Build history of the part. All positions in model axes, mm. A direction names the side the tool comes from. Round coordinates to 2 decimals unless told otherwise and drop trailing zeros. Write each loop counter-clockwise with the first axis right and the second up, starting at its lowest first coordinate (ties: lowest second). Pieces come first, ordered by that corner, then holes. Notation, with made-up numbers: (20, 24.25) - (79, 24.25) arc R28 cw to (79, 55.25) - close; hole circle Ø1 at (44.5, 45.5). An arc over 180 degrees is marked (long way). Answer as a JSON object with one key per item and string values. Group by question number.
Item 1: Flat gauge pins, fed straight in: pin 1 (2 mm diameter, centred on x = 25, y = -3.5, fed in from +Z); pin 2 (6 mm diameter, centred on x = 2, y = -5.5, fed in from +Z); pin 3 (4 mm diameter, centred on x = -4, z = 22.5, fed in from +Y); pin 4 (1.5 mm diameter, centred on y = -5, z = 26, fed in from -X). Where does each tip first touch, or does it go through?
Item 2: Slice it at D-D, the plane x = -9.5. List the corners of the cut face in (y, z), then the cut area to 3 significant figures.
Item 3: Slice it at C-C, the plane x = -39. List the corners of the cut face in (y, z).
Item 4: Slice it at A-A, the plane z = 2. List the corners of the cut face in (x, y), then the cut area to 3 significant figures.
Item 5: Two-plate mould, pull along X, no slides. Class faces 5 (the flat face through (43, 0, 0)), 6 (the flat face through (41.15, 0, 0)), 7 (the cylindrical face through (-0.867, -3.905, 17.853)): +X half, -X half, draft (parallel to the pull), parting line (faces both ways), or undercut.
Item 6: Slice it at B-B, the plane y = 0. List the corners of the cut face in (x, z).
Item 7: Which spindle directions (+Z, -Z, +X, -X, +Y, -Y) get a long thin tool onto all of the face, cutting with end or side? Do faces 1 (the cylindrical face through (39.05, 7.15, -0.08)), 2 (the cylindrical face through (-0.867, -3.905, 29.993)), 3 (the cylindrical face through (3.796, -0.167, 28.993)), 4 (the flat face through (-1, -12, 0)). Say none if no direction does.
Item 8: Probe line 1 (Z direction, x = 18.5, y = -8); line 2 (X direction, y = 5, z = 6.5); line 3 (X direction, y = 2.5, z = 8). List the from-to ranges inside material, lowest first. Write a range as from..to.
from build123d import *

# Parameters (mm, degrees)
SKETCH_1_W          = 86
SKETCH_1_H          = 24
EXTRUDE_1_DEPTH     = 5.5
SKETCH_2_R          = 4
EXTRUDE_2_DEPTH     = 3.5
SKETCH_3_R          = 4
EXTRUDE_3_DEPTH     = 21.5
CUT_EXTRUDE_4_DEPTH = 58.349803836
SKETCH_15_R         = 4
CUT_EXTRUDE_5_DEPTH = 9.999
SKETCH_4_W          = 0.2
SKETCH_4_H          = 1
SKETCH_16_R         = 2.9995
EXTRUDE_4_DEPTH     = 8.999
SKETCH_18_R         = 6
EXTRUDE_5_DEPTH     = 2
SKETCH_22_R         = 7.5
EXTRUDE_7_DEPTH     = 11
CHAMFER_1_SIZE      = 1


with BuildPart() as part:
    # 草图1 → 凸台-拉伸1 (new, symmetric)
    with BuildSketch(Plane.XY):
        Rectangle(SKETCH_1_W, SKETCH_1_H)
    extrude(amount=EXTRUDE_1_DEPTH, both=True)

    # 草图2 → 凸台-拉伸2 (add)
    with BuildSketch(Plane.XY.offset(5.5)):
        Circle(SKETCH_2_R)
    extrude(amount=EXTRUDE_2_DEPTH)

    # 草图3 → 凸台-拉伸3 (add)
    with BuildSketch(Plane.XY.offset(9)):
        Circle(SKETCH_3_R)
    extrude(amount=EXTRUDE_3_DEPTH)

    # 草图14 → 切除-拉伸4 (cut, through all)
    with BuildSketch(Plane(origin=(0, 0, -5.5), x_dir=(-1, 0, 0), z_dir=(0, 0, -1))):
        with BuildLine():
            Line((-36.85, 5), (-36.85, -5))
            ThreePointArc((-36.85, -5), (-39, -7.15), (-41.15, -5))
            Line((-41.15, -5), (-41.15, 5))
            ThreePointArc((-41.15, 5), (-39, 7.15), (-36.85, 5))
        make_face()
        with BuildLine():
            Line((36.85, 5), (36.85, -5))
            ThreePointArc((36.85, -5), (39, -7.15), (41.15, -5))
            Line((41.15, -5), (41.15, 5))
            ThreePointArc((41.15, 5), (39, 7.15), (36.85, 5))
        make_face()
    extrude(amount=-CUT_EXTRUDE_4_DEPTH, mode=Mode.SUBTRACT)

    # 草图15 → 切除-拉伸5 (cut)
    with BuildSketch(Plane(origin=(0, 0, -5.5), x_dir=(-1, 0, 0), z_dir=(0, 0, -1))):
        with Locations(Location((0, 0, 0), (0, 0, 180))):
            Circle(SKETCH_15_R)
    extrude(amount=-CUT_EXTRUDE_5_DEPTH, mode=Mode.SUBTRACT)

    # 草图4 → 切除-旋转1 (revolve, cut)
    with BuildSketch(Plane(origin=(0, 0, 0), x_dir=(1, 0, 0), z_dir=(0, 1, 0))):
        with Locations((-3.9, -29)):
            Rectangle(SKETCH_4_W, SKETCH_4_H)
    revolve(axis=Axis((0, 0, 0), (0, 0, 1)), mode=Mode.SUBTRACT)

    # 草图16 → 凸台-拉伸4 (add)
    with BuildSketch(Plane(origin=(0, 0, 4.499), x_dir=(-1, 0, 0), z_dir=(0, 0, -1))):
        Circle(SKETCH_16_R)
    extrude(amount=EXTRUDE_4_DEPTH)

    # 草图18 → 凸台-拉伸5 (add)
    with BuildSketch(Plane.XY.offset(5.5)):
        Circle(SKETCH_18_R)
    extrude(amount=EXTRUDE_5_DEPTH)

    # 草图22 → 凸台-拉伸7 (add)
    with BuildSketch(Plane(origin=(0, 0, -5.5), x_dir=(-1, 0, 0), z_dir=(0, 0, -1))):
        Circle(SKETCH_22_R)
    extrude(amount=-EXTRUDE_7_DEPTH)

    # 倒角1
    chamfer_1_edges = [part.edges().sort_by_distance(p)[0] for p in [
        (43, -12, 0),
        (-43, -12, 0),
        (-43, 12, 0),
        (43, 12, 0),
    ]]
    chamfer(chamfer_1_edges, length=CHAMFER_1_SIZE)


solid = part.part
Geometry says:
{
 "1": {"pin 1": "stops at z = 5.5", "pin 2": "stops at z = 30.5", "pin 3": "stops at y = 3.46", "pin 4": "passes through"},
 "2": {"outline": "(-12, -5.5) - (12, -5.5) - (12, 5.5) - (-12, 5.5) - close", "area": "264 mm^2"},
 "3": {"outline": "(-12, -5.5) - (-7.15, -5.5) - (-7.15, 5.5) - (-12, 5.5) - close; (7.15, -5.5) - (12, -5.5) - (12, 5.5) - (7.15, 5.5) - close"},
 "4": {"outline": "(-43, -11) - (-42, -12) - (42, -12) - (43, -11) - (43, 11) - (42, 12) - (-42, 12) - (-43, 11) - close; hole (-41.15, -5) arc R2.15 ccw to (-36.85, -5) - (-36.85, 5) arc R2.15 ccw to (-41.15, 5) - close; hole (36.85, -5) arc R2.15 ccw to (41.15, -5) - (41.15, 5) arc R2.15 ccw to (36.85, 5) - close", "area": "1,950 mm^2"},
 "5": {"face 5": "+X half", "face 6": "undercut", "face 7": "parting line"},
 "6": {"outline": "(-43, -5.5) - (-41.15, -5.5) - (-41.15, 5.5) - (-43, 5.5) - close; (-36.85, -5.5) - (36.85, -5.5) - (36.85, 5.5) - (6, 5.5) - (6, 7.5) - (4, 7.5) - (4, 28.5) - (3.8, 28.5) - (3.8, 29.5) - (4, 29.5) - (4, 30.5) - (-4, 30.5) - (-4, 29.5) - (-3.8, 29.5) - (-3.8, 28.5) - (-4, 28.5) - (-4, 7.5) - (-6, 7.5) - (-6, 5.5) - (-36.85, 5.5) - close; (41.15, -5.5) - (43, -5.5) - (43, 5.5) - (41.15, 5.5) - close"},
 "7": {"face 1": "+Z, -Z", "face 2": "+Z", "face 3": "none", "face 4": "+Z, -Z, +X, -X, -Y"},
 "8": {"line 1": "z = -5.5..5.5", "line 2": "x = -3.32..3.32", "line 3": "x = -3.12..3.12"}
}
